from build123d import *

# Parameters (mm, degrees)
SKETCH_1_W                = 150
SKETCH_1_H                = 70
EXTRUDE_1_DEPTH           = 15
HOLE_WIZARD_1_D           = 9
HOLE_WIZARD_1_CBORE_D     = 15
HOLE_WIZARD_1_CBORE_DEPTH = 9
HOLE_WIZARD_12_5_12_5_1_D = 12.5


with BuildPart() as part:
    # 草图1 → 凸台-拉伸1 (new body)
    with BuildSketch(Plane(origin=(0, 0, 0), x_dir=(0, 0, -1), z_dir=(1, 0, 0))):
        Rectangle(SKETCH_1_W, SKETCH_1_H)
    extrude(amount=EXTRUDE_1_DEPTH)

    # 打孔尺寸(%根据)内六角圆柱头螺钉的类型1 (through all)
    with Locations(Plane(origin=(15, 0, 0), x_dir=(0, 0, -1), z_dir=(1, 0, 0))):
        with Locations((-24, 24), (24, 24), (-24, -24), (24, -24)):
            CounterBoreHole(HOLE_WIZARD_1_D / 2, HOLE_WIZARD_1_CBORE_D / 2, HOLE_WIZARD_1_CBORE_DEPTH)

    # Ø12.5 (12.5) 直径孔1 (through all)
    with Locations(Plane.ZY):
        with Locations((-60, 20), (-60, -20), (60, 20), (60, -20)):
            Hole(HOLE_WIZARD_12_5_12_5_1_D / 2)


solid = part.part
Design review of the part built by this model. Coordinates are the model's own, in mm. A direction names the side the tool comes from. Round coordinates to 2 decimals unless told otherwise and drop trailing zeros. Loops run counter-clockwise (first coordinate to the right, second up) from the corner with the lowest first, then second, coordinate; pieces in that order, holes last. Notation, with made-up numbers: (-1, 8.5) - (4, 8.5) arc R33 ccw to (4, 39.5) - close; hole circle Ø9 at (52, 38.25). An arc over 180 degrees is marked (long way). One line per question, with ' | ' between items.
1. Clearance check with flat-ended pins moving along their axes: P1, Ø7.5, axis at y = 20, z = 60, coming from the +X side; P2, Ø11.5, axis at y = 24, z = -24, coming from the +X side. State where each tip first meets the part, or that it passes through.
Results are:
P1: passes through | P2: stops at x = 6
2. We need section B-B, the plane x = 4. State how many separate pieces and enclosed holes the cut face has, and give its area (3 significant figures).
Results are:
separate pieces: 1 | enclosed holes: 8 | area: 9,750 mm²
3. We need section A-A, the plane z = -60. State the section outline as (x, y) points.
Results are:
outline: (0, -35) - (15, -35) - (15, -26.25) - (0, -26.25) - close; (0, -13.75) - (15, -13.75) - (15, 13.75) - (0, 13.75) - close; (0, 26.25) - (15, 26.25) - (15, 35) - (0, 35) - close
4. Draft analysis for pull direction Z (two halves, no side actions). For faces 3 (the face through (0, 0, 1)), 4 (the face through (7, 0, 75)), 5 (the face through (6, -24, 19)), state which applies: released by +Z, released by -Z, zero draft, split by the parting line, or undercut.
Results are:
face 3: zero draft | face 4: released by +Z | face 5: undercut
5. We need section D-D, the plane z = -24. State the section outline as (x, y) points, and give its area (3 significant figures).
Results are:
outline: (0, -35) - (15, -35) - (15, -31.5) - (6, -31.5) - (6, -28.5) - (0, -28.5) - close; (0, -19.5) - (6, -19.5) - (6, -16.5) - (15, -16.5) - (15, 16.5) - (6, 16.5) - (6, 19.5) - (0, 19.5) - close; (0, 28.5) - (6, 28.5) - (6, 31.5) - (15, 31.5) - (15, 35) - (0, 35) - close | area: 672 mm²
6. For faces 1 (the face through (6, 24, 19)), 2 (the face through (7.6, 21.88, 54.04)), list the 3-axis set-ups (+Z, -Z, +X, -X, +Y, -Y) from which the entire face can be reached by the end or side of a thin tool; tool diameter is ignored.
Results are:
face 1: +X | face 2: +X, -X
7. For L1, parallel to Y at x = 5, z = 60; L2, parallel to Y at x = 4.5, z = -24; L3, parallel to Z at x = 7, y = 25.5, list the stretches that pass through material, from the lowest coordinate up. Write a range as [from, to].
Results are:
L1: y = [-35, -26.25], [-13.75, 13.75], [26.25, 35] | L2: y = [-35, -28.5], [-19.5, 19.5], [28.5, 35] | L3: z = [-75, -62.97], [-57.03, -31.35], [-16.65, 16.65], [31.35, 57.03], [62.97, 75]
8. We need section C-C, the plane y = -24. State the section outline as (x, z) points, and give its area (3 significant figures).
Results are:
outline: (0, -75) - (15, -75) - (15, -64.8) - (0, -64.8) - close; (0, -55.2) - (15, -55.2) - (15, -31.5) - (6, -31.5) - (6, -28.5) - (0, -28.5) - close; (0, -19.5) - (6, -19.5) - (6, -16.5) - (15, -16.5) - (15, 16.5) - (6, 16.5) - (6, 19.5) - (0, 19.5) - close; (0, 28.5) - (6, 28.5) - (6, 31.5) - (15, 31.5) - (15, 55.2) - (0, 55.2) - close; (0, 64.8) - (15, 64.8) - (15, 75) - (0, 75) - close | area: 1,580 mm²
